Model file for the job. Use its own axes, mm. Round coordinates to 2 decimals unless told otherwise and drop trailing zeros. Write each loop counter-clockwise with the first axis right and the second up, starting at its lowest first coordinate (ties: lowest second). Pieces come first, ordered by that corner, then holes.
```python
from build123d import *

# Parameters (mm, degrees)
SKETCH1_W              = 80
SKETCH1_H              = 80
BOSS_EXTRUDE1_DEPTH    = 30
FILLET1_R              = 5
M24X2_0_TAPPED_HOLE1_D = 22


with BuildPart() as part:
    # Sketch1 → Boss-Extrude1 (new body)
    with BuildSketch(Plane(origin=(0, 0, 0), x_dir=(1, 0, 0), z_dir=(0, 1, 0))):
        Rectangle(SKETCH1_W, SKETCH1_H)
    extrude(amount=BOSS_EXTRUDE1_DEPTH)

    # Fillet1
    fillet1_edges = [part.edges().sort_by_distance(p)[0] for p in [
        (40, 15, 40),
        (-40, 15, 40),
        (-40, 15, -40),
        (40, 15, -40),
    ]]
    fillet(fillet1_edges, radius=FILLET1_R)

    # M24x2.0 Tapped Hole1 (through all)
    with Locations(Plane(origin=(0, 30, 0), x_dir=(1, 0, 0), z_dir=(0, 1, 0))):
        with Locations((0, 0)):
            Hole(M24X2_0_TAPPED_HOLE1_D / 2)


solid = part.part
```
1) Cut at C-C on x = 1. List the corners of the cut face in (y, z).
2) Cut at A-A on z = 0. List the corners of the cut face in (x, y).
3) Pull direction Z, two halves, no side cores. Call faces 1 (the face through (2.38, 14.79, 10.74)), 2 (the face through (-39, 15, -38)), 3 (the face through (-9, 30, 8)): released by +Z, released by -Z, zero draft, split by the parting line, or undercut.
4) Flat gauge pin, fed straight in: pin 1 Ø10 at (x, z) = (22, -26.5) entering from -Y. Where does the tip first touch, or does it go through?
5) Cut at B-B on y = 11. List the corners of the cut face in (x, z).
6) Wall check: probe 1 along Z at (x, y) = (0, 13); probe 2 along Z at (x, y) = (5, 18); probe 3 along X at (y, z) = (26.25, -2.5). Give the ranges that are in metal, low to high.
Result sheet:
1. outline: (0, -40) - (30, -40) - (30, -10.95) - (0, -10.95) - close; (0, 10.95) - (30, 10.95) - (30, 40) - (0, 40) - close
2. outline: (-40, 0) - (-11, 0) - (-11, 30) - (-40, 30) - close; (11, 0) - (40, 0) - (40, 30) - (11, 30) - close
3. face 1: undercut
3. face 2: released by -Z
3. face 3: zero draft
4. pin 1: stops at y = 0
5. outline: (-40, -35) arc R5 ccw to (-35, -40) - (35, -40) arc R5 ccw to (40, -35) - (40, 35) arc R5 ccw to (35, 40) - (-35, 40) arc R5 ccw to (-40, 35) - close; hole circle Ø22 at (0, 0)
6. probe 1: z = -40 to -11, 11 to 40
6. probe 2: z = -40 to -9.8, 9.8 to 40
6. probe 3: x = -40 to -10.71, 10.71 to 40
